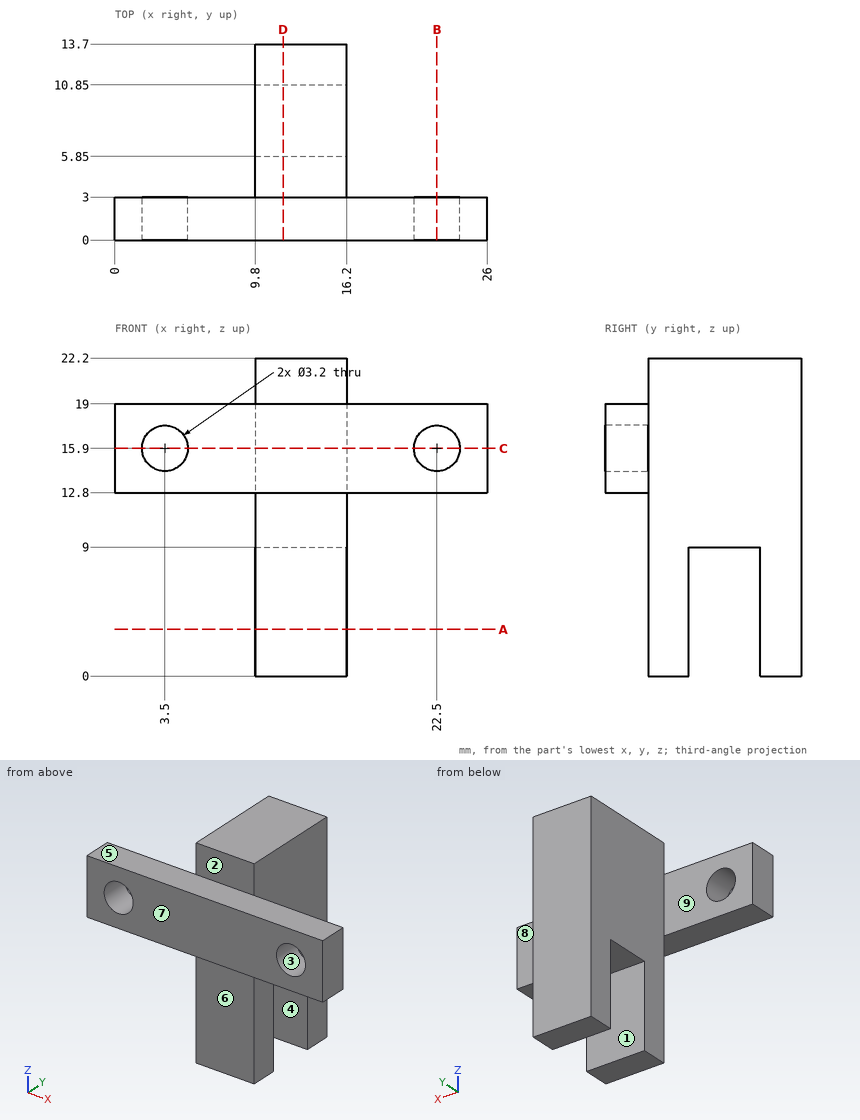
The figure shows three views and two pictorial views of one solid part (mm, origin at its lowest corner). Answer the questions. A direction names the side the tool comes from. Round coordinates to 2 decimals unless told otherwise and drop trailing zeros. Write each loop counter-clockwise with the first axis right and the second up, starting at its lowest first coordinate (ties: lowest second). Pieces come first, ordered by that corner, then holes. Notation, with made-up numbers: (6.5, -31.5) -> (39.5, -31.5) arc R34 cw to (39.5, 3.5) -> close; hole circle Ø1 at (3, 23.25). An arc over 180 degrees is marked (long way). Write each question's results on one line, items separated by ' | '.
Q1. Flat-ended cylindrical pins translate along their axes: P1, Ø4, axis at x = 6, y = 4, coming from the +Z side; P2, Ø3, axis at x = 18.5, y = 3, coming from the -Z side; P3, Ø5, axis at x = 4.5, z = 16, coming from the +Y side. Find the tip coordinate at first contact, or state that the pin passes through.
Data:
P1: z = 19 | P2: z = 12.8 | P3: y = 3
Q2. Section D-D, the plane x = 11.75 is taken. Write down the section's boundary in (y, z), then the cut area to 3 significant figures.
Data:
outline: (0, 12.8) -> (3, 12.8) -> (3, 0) -> (5.85, 0) -> (5.85, 9) -> (10.85, 9) -> (10.85, 0) -> (13.7, 0) -> (13.7, 22.2) -> (3, 22.2) -> (3, 19) -> (0, 19) -> close | area: 211 mm^2
Q3. Determine the mould class of the marked faces 1, 2, 3 and 4 for opening direction Y: released by +Y, released by -Y, zero draft, split by the parting line, or undercut.
Data:
face 1: undercut | face 2: released by -Y | face 3: zero draft | face 4: undercut
Q4. Section B-B, the plane x = 22.5 is taken. Write down the section's boundary in (y, z), then the cut area to 3 significant figures.
Data:
outline: (0, 12.8) -> (3, 12.8) -> (3, 14.3) -> (0, 14.3) -> close; (0, 17.5) -> (3, 17.5) -> (3, 19) -> (0, 19) -> close | area: 9.00 mm^2
Q5. Section C-C, the plane z = 15.9 is taken. Write down the section's boundary in (x, y), then the cut area to 3 significant figures.
Data:
outline: (0, 0) -> (1.9, 0) -> (1.9, 3) -> (0, 3) -> close; (5.1, 0) -> (20.9, 0) -> (20.9, 3) -> (16.2, 3) -> (16.2, 13.7) -> (9.8, 13.7) -> (9.8, 3) -> (5.1, 3) -> close; (24.1, 0) -> (26, 0) -> (26, 3) -> (24.1, 3) -> close | area: 127 mm^2
Q6. Straight lines are drawn through the part: line 1 along X through (y, z) = (0.9, 15.9); line 2 along X through (y, z) = (2.5, 17.25); line 3 along Y through (x, z) = (11.5, 7). For each, find the intervals that lie inside material, in ascending order. Write a range as [from, to].
Data:
line 1: [0, 1.9], [5.1, 20.9], [24.1, 26] | line 2: [0, 2.64], [4.36, 21.64], [23.36, 26] | line 3: [3, 5.85], [10.85, 13.7]
Q7. Section A-A, the plane z = 3.25 is taken. Write down the section's boundary in (x, y).
Data:
outline: (9.8, 3) -> (16.2, 3) -> (16.2, 5.85) -> (9.8, 5.85) -> close; (9.8, 10.85) -> (16.2, 10.85) -> (16.2, 13.7) -> (9.8, 13.7) -> close
Q8. Which of the six approach directions +Z, -Z, +X, -X, +Y, -Y give full straight-line access (tool end or side, diameter ignored) to the marked faces 5, 6, 7, 8 and 9?
Data:
face 5: +Z, +X, -X, -Y | face 6: -Z, +X, -X, -Y | face 7: +Z, -Z, +X, -X, -Y | face 8: +Z, -Z, +X, +Y | face 9: +Z, -Z, -X, +Y
